CAD build for the part. Positions are in the model's coordinates, mm. A direction names the side the tool comes from. Give positions to 0.01 mm unless a question says otherwise; leave off trailing zeros. Write each loop counter-clockwise with the first axis right and the second up, starting at its lowest first coordinate (ties: lowest second). Pieces come first, ordered by that corner, then holes. Notation, with made-up numbers: (-11, -30) -> (46, -30) arc R14 ccw to (46, -25) -> close; hole circle Ø7 at (77.25, 68.25). An arc over 180 degrees is marked (long way). Answer in a Markdown table with one row per item. Add a question column.
```python
from build123d import *

# Parameters (mm, degrees)
SKETCH1_W           = 94
SKETCH1_H           = 24
BOSS_EXTRUDE1_DEPTH = 18
SKETCH2_W           = 36
SKETCH2_H           = 10
CUT_EXTRUDE1_DEPTH  = 70
CHAMFER1_SIZE       = 3.5
CHAMFER2_SIZE       = 3.5
SKETCH3_R           = 3
CUT_EXTRUDE2_DEPTH  = 70


with BuildPart() as part:
    # Sketch1 → Boss-Extrude1 (new body)
    with BuildSketch(Plane(origin=(0, 0, 0), x_dir=(1, 0, 0), z_dir=(0, 1, 0))):
        Rectangle(SKETCH1_W, SKETCH1_H)
    extrude(amount=BOSS_EXTRUDE1_DEPTH)

    # Sketch2 → Cut-Extrude1 (cut)
    with BuildSketch(Plane(origin=(0, 18, 0), x_dir=(1, 0, 0), z_dir=(0, 1, 0))):
        with Locations((-47, 0)):
            Rectangle(SKETCH2_W, SKETCH2_H)
        with Locations((47, 0)):
            Rectangle(SKETCH2_W, SKETCH2_H)
    extrude(amount=-CUT_EXTRUDE1_DEPTH, mode=Mode.SUBTRACT)

    # Chamfer1
    chamfer1_edges = [part.edges().sort_by_distance(p)[0] for p in [
        (47, 18, -8.5),
        (47, 18, 8.5),
    ]]
    chamfer(chamfer1_edges, length=CHAMFER1_SIZE)

    # Chamfer2
    chamfer2_edges = [part.edges().sort_by_distance(p)[0] for p in [
        (-47, 18, -8.5),
        (-47, 0, 8.5),
        (-47, 18, 8.5),
        (-47, 0, -8.5),
    ]]
    chamfer(chamfer2_edges, length=CHAMFER2_SIZE)

    # Sketch3 → Cut-Extrude2 (cut)
    with BuildSketch(Plane.XY.offset(12)):
        with Locations((-40, 9)):
            Circle(SKETCH3_R)
    extrude(amount=-CUT_EXTRUDE2_DEPTH, mode=Mode.SUBTRACT)


solid = part.part
```
Item 1: Slice it at A-A, the plane y = 9. List the corners of the cut face in (x, z), then the cut area to 3 significant figures.
Item 2: Probe L1, parallel to Y at x = -40, z = -6.5; L2, parallel to Z at x = -39, y = 14.25; L3, parallel to X at y = 14.5, z = -0.5. List the from-to ranges inside material, lowest first. Write a range as from..to.
Item 3: Mould opens along X. For faces 1 (the face through (-43, 9, 9)), 2 (the face through (-29, 9, 0)), 3 (the face through (-1, 9, -12)), 4 (the face through (47, 7, 9)) say: released by +X, released by -X, zero draft, split by the parting line, or undercut.
Item 4: Slice it at C-C, the plane z = 8. List the corners of the cut face in (x, y), then the cut area to 3 significant figures.
Item 5: Drop flat-ended pins along their axis: pin 1 Ø2 at (y, z) = (12, -3) entering from -X; pin 2 Ø3 at (y, z) = (10, 0) entering from +X; pin 3 Ø1.5 at (x, z) = (-33, -3.5) entering from +Y. Give the stop position or say it passes through.
Item 6: Slice it at D-D, the plane y = 17. List the corners of the cut face in (x, z), then the cut area to 3 significant figures.
Item 7: Slice it at B-B, the plane x = -40. List the corners of the cut face in (y, z).
Item 8: Which spindle directions (+Z, -Z, +X, -X, +Y, -Y) get a long thin tool onto all of the face, cutting with end or side? Do faces 5 (the face through (1, 0, 0)), 6 (the face through (38, 9, 5)). Say none if no direction does.
Answer key:
| question | item | result |
|---|---|---|
| 1 | outline | (-47, -12) -> (-43, -12) -> (-43, -5) -> (-47, -5) -> close; (-47, 5) -> (-43, 5) -> (-43, 12) -> (-47, 12) -> close; (-37, -12) -> (47, -12) -> (47, -5) -> (29, -5) -> (29, 5) -> (47, 5) -> (47, 12) -> (-37, 12) -> (-37, 5) -> (-29, 5) -> (-29, -5) -> (-37, -5) -> close |
| 1 | area | 1,810 mm² |
| 2 | L1 | y = 0..6, 12..18 |
| 2 | L2 | z = -12..-5, 5..12 |
| 2 | L3 | x = -29..29 |
| 3 | face 1 | undercut |
| 3 | face 2 | released by -X |
| 3 | face 3 | zero draft |
| 3 | face 4 | released by +X |
| 4 | outline | (-47, 3.5) -> (-43.5, 0) -> (47, 0) -> (47, 14.5) -> (43.5, 18) -> (-43.5, 18) -> (-47, 14.5) -> close; hole circle Ø6 at (-40, 9) |
| 4 | area | 1,650 mm² |
| 5 | pin 1 | stops at x = -29 |
| 5 | pin 2 | stops at x = 29 |
| 5 | pin 3 | passes through |
| 6 | outline | (-44.5, -12) -> (44.5, -12) -> (44.5, -5) -> (29, -5) -> (29, 5) -> (44.5, 5) -> (44.5, 12) -> (-44.5, 12) -> (-44.5, 5) -> (-29, 5) -> (-29, -5) -> (-44.5, -5) -> close |
| 6 | area | 1,830 mm² |
| 7 | outline | (0, -12) -> (6, -12) -> (6, -5) -> (0, -5) -> close; (0, 5) -> (6, 5) -> (6, 12) -> (0, 12) -> close; (12, -12) -> (18, -12) -> (18, -5) -> (12, -5) -> close; (12, 5) -> (18, 5) -> (18, 12) -> (12, 12) -> close |
| 8 | face 5 | +Z, -Z, +X, -X, -Y |
| 8 | face 6 | +X, +Y, -Y |
